Verification items for the finished model (mm, model axes). Face numbers are marked on the shaded views. Round coordinates to 2 decimals unless told otherwise and drop trailing zeros. Write each loop counter-clockwise with the first axis right and the second up, starting at its lowest first coordinate (ties: lowest second). Pieces come first, ordered by that corner, then holes. Notation, with made-up numbers: M -22.75,74 L -7.75,74 A15 ccw -7.75,101 Z; hole C 47,52.5 d2. An arc over 180 degrees is marked long. One line per item, written item: value. Start each with the question number.
from build123d import *

# Parameters (mm, degrees)
SKETCH1_R           = 5
BOSS_EXTRUDE1_DEPTH = 10


with BuildPart() as part:
    # Sketch1 → Boss-Extrude1 (new body)
    with BuildSketch(Plane.XY):
        with BuildLine():
            Line((-35, -40), (35, -40))
            Line((35, -40), (8.630305493, 5.051517306))
            ThreePointArc((8.630305493, 5.051517306), (0, 10), (-8.630305493, 5.051517306))
            Line((-8.630305493, 5.051517306), (-35, -40))
        make_face()
        Circle(SKETCH1_R, mode=Mode.SUBTRACT)
    extrude(amount=BOSS_EXTRUDE1_DEPTH)


solid = part.part
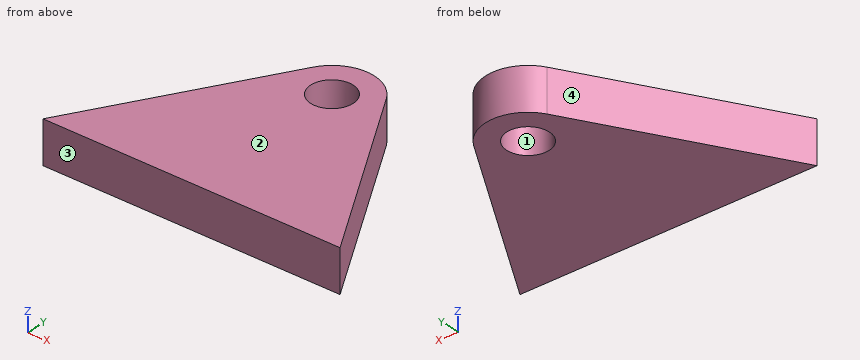
1) Cross-section at A-A (x = 0). Record the boundary of the cut face in (y, z).
2) Thickness scan on line 1 (Y direction, x = 0, z = 5.25); line 2 (X direction, y = -21, z = 9.75); line 3 (X direction, y = -13, z = 3). Record the ranges inside material, lowest first.
3) Cross-section at C-C (y = 0). Record the boundary of the cut face in (x, z), then the cut area to 3 significant figures.
4) Cross-section at D-D (y = -30). Record the boundary of the cut face in (x, z), then the cut area to 3 significant figures.
5) Mould release check, pull along Y, two halves, no side actions. Record for the marked faces 1, 2, 3 and 4: pulls with the +Y half, pulls with the -Y half, needs draft (parallel to the pull), parting line crosses it, or undercut.
6) Cross-section at B-B (z = 5.5). Record the boundary of the cut face in (x, y), then the cut area to 3 significant figures.
7) Gauge pin test, flat ends, axial feed: pin 1 Ø4 at (x, z) = (-21.5, 1.5) entering from +Y; pin 2 Ø1 at (x, z) = (-23.5, 8) entering from +Y; pin 3 Ø3 at (y, z) = (-17, 6) entering from +X. Record the tip position at first contact, or that the pin passes through.
Results below:
1. outline: M -40,0 L -5,0 L -5,10 L -40,10 Z; M 5,0 L 10,0 L 10,10 L 5,10 Z
2. line 1: y = -40 to -5, 5 to 10
2. line 2: x = -23.88 to 23.88
2. line 3: x = -19.2 to 19.2
3. outline: M -11.59,0 L -5,0 L -5,10 L -11.59,10 Z; M 5,0 L 11.59,0 L 11.59,10 L 5,10 Z
3. area: 132 mm²
4. outline: M -29.15,0 L 29.15,0 L 29.15,10 L -29.15,10 Z
4. area: 583 mm²
5. face 1: undercut
5. face 2: needs draft
5. face 3: pulls with the -Y half
5. face 4: pulls with the +Y half
6. outline: M -35,-40 L 35,-40 L 8.63,5.05 A10 ccw -8.63,5.05 Z; hole C 0,0 d10
6. area: 1,950 mm²
7. pin 1: stops at y = -13.52
7. pin 2: stops at y = -19.5
7. pin 3: stops at x = 22.42
